Can you work these out from the model? Positions are in its coordinate system, mm. A direction names the side the tool comes from. Coordinates: 2 decimals unless noted, no trailing zeros. Loops run counter-clockwise (first coordinate to the right, second up) from the corner with the lowest first, then second, coordinate; pieces in that order, holes last. Notation, with made-up numbers: (-15, -24.5) -> (40, -24.5) arc R27 cw to (40, -4.5) -> close; hole circle Ø7 at (56, -4.75). An arc over 180 degrees is marked (long way). Use one line per item in the form item = value. Start each with the question number.
(1) Imagine slicing it at C-C (y = 80). List the corners of the cut face in (x, z) for me, plus the area to 3 significant figures.
(2) I need wall thicknesses on line 1 (Z direction, x = 0, y = 105); line 2 (Y direction, x = -30.5, z = 21); line 3 (Z direction, x = -128, y = -83). Which ranges of each line are inside material? Lowest first, please. Write a range as [from, to].
(3) I'm going to push flat-ended pins straight in: pin 1 (3 mm diameter, centred on x = -124, y = 54, fed in from +Z); pin 2 (3 mm diameter, centred on x = -59, z = 40.5, fed in from -Y); pin 3 (2 mm diameter, centred on x = 159, y = -63.5, fed in from +Z). Where does each tip first touch, or does it pass through?
(4) Imagine slicing it at B-B (z = 30). List the corners of the cut face in (x, y) for me, plus the area to 3 significant figures.
(5) On a 3-axis mill with a long thin cutter (end or side, diameter ignored), from which of +Z, -Z, +X, -X, +Y, -Y can I reach the whole of each face in a straight line? I mean faces 1 (the flat face through (-3, -29, 10)), 2 (the flat face through (-1, 107.5, 33)). Say none if no direction works.
(6) Imagine slicing it at A-A (x = -18.5). List the corners of the cut face in (y, z) for me, plus the area to 3 significant figures.
```python
from build123d import *

# Parameters (mm, degrees)
SKETCH_1_W             = 404
SKETCH_1_H             = 215
EXTRUDE_1_DEPTH        = 70
SHELL_1_T              = -10
CUT_EXTRUDE_1_DEPTH    = 80
SKETCH_6_W             = 881.925411548
SKETCH_6_H             = 167.715249963
CUT_EXTRUDE_2_DEPTH    = 205
HOLE_WIZARD_M8_1_D     = 6.8
HOLE_WIZARD_M8_1_DEPTH = 19.75
HOLE_WIZARD_M8_1_TIP   = 2.042926105
FILLET_1_R             = 10


with BuildPart() as part:
    # 草图1 → 凸台-拉伸1 (new body)
    with BuildSketch(Plane.XY):
        Rectangle(SKETCH_1_W, SKETCH_1_H)
    extrude(amount=EXTRUDE_1_DEPTH)

    # 抽壳1
    shell_1_openings = [part.faces().sort_by_distance(p)[0] for p in [
        (-202, 0, 35),
        (202, 0, 35),
    ]]
    offset(amount=SHELL_1_T, openings=shell_1_openings, kind=Kind.INTERSECTION)

    # 草图2 → 切除-拉伸1 (cut)
    with BuildSketch(Plane.XY.offset(70)):
        Polygon((-202, -86.489690448), (-90, 107.5), (-202, 107.5), align=None)
        Polygon((90, 107.5), (202, 107.5), (202, -86.489690448), align=None)
    extrude(amount=-CUT_EXTRUDE_1_DEPTH, mode=Mode.SUBTRACT)

    # 草图6 → 切除-拉伸2 (cut)
    with BuildSketch(Plane.XZ.offset(107.5)):
        with Locations((-202, 93.857624982)):
            Rectangle(SKETCH_6_W, SKETCH_6_H)
    extrude(amount=-CUT_EXTRUDE_2_DEPTH, mode=Mode.SUBTRACT)

    # M8 螺纹孔1
    with Locations(Plane(origin=(0, 107.5, 0), x_dir=(1, 0, 0), z_dir=(0, 1, 0))):
        with Locations((-50, -40), (0, -40), (50, -40)):
            Hole(HOLE_WIZARD_M8_1_D / 2, depth=HOLE_WIZARD_M8_1_DEPTH)
            with Locations((0, 0, -(HOLE_WIZARD_M8_1_DEPTH + HOLE_WIZARD_M8_1_TIP / 2))):  # 118° drill point
                Cone(0, HOLE_WIZARD_M8_1_D / 2, HOLE_WIZARD_M8_1_TIP, mode=Mode.SUBTRACT)

    # 圆角1
    fillet_1_edges = [part.edges().sort_by_distance(p)[0] for p in [
        (0, 107.5, 0),
        (92.886751346, 102.5, 70),
        (-92.886751346, 102.5, 70),
    ]]
    fillet(fillet_1_edges, radius=FILLET_1_R)


solid = part.part
```
Worked out:
q1.outline = (-105.88, 0) -> (105.88, 0) -> (105.88, 10) -> (-105.88, 10) -> close
q1.area = 2,120 mm2
q2.line_1 = [3.39, 36.6], [43.4, 70]
q2.line_2 = [97.5, 107.5]
q2.line_3 = [0, 10]
q3.pin_1 = through
q3.pin_2 = 97.5
q3.pin_3 = 10
q4.outline = (-95.77, 97.5) -> (95.77, 97.5) -> (90, 107.5) -> (-90, 107.5) -> close
q4.area = 1,860 mm2
q5.face_1 = +Z, +X, -X, -Y
q5.face_2 = +Z, -Z, +X, -X, +Y
q6.outline = (-107.5, 0) -> (97.5, 0) arc R10 ccw to (107.5, 10) -> (107.5, 70) -> (97.5, 70) -> (97.5, 10) -> (-107.5, 10) -> close
q6.area = 2,730 mm2
